Answer from the drawing. Dimensions are ordinates in mm from the lowest x, y and z of the part. A direction names the side the tool comes from. Coordinates: 2 decimals unless noted, no trailing zeros. Write each loop counter-clockwise with the first axis right and the second up, starting at its lowest first coordinate (ties: lowest second). Pieces come first, ordered by that corner, then holes.
1) Find the intervals of material crossed by line 1 (Y direction, x = 10, z = 26) (1 decimal); line 2 (Y direction, x = 1.5, z = 32); line 3 (Y direction, x = 12, z = 26), in increasing order.
2) The part is cut by section B-B (z = 20.5). Determine the outline of the cut face in (x, y) (1 decimal).
3) The part is cut by section A-A (x = 10). Determine the outline of the cut face in (y, z) (1 decimal).
4) Determine the mould class of the marked faces 1, 2, 3 and 4 for opening direction X: +X half, -X half, draft (parallel to the pull), parting line (faces both ways), or undercut.
5) Which of the six approach directions +Z, -Z, +X, -X, +Y, -Y give full straight-line access (tool end or side, diameter ignored) to the marked faces 5 and 6?
6) Each of these flat-tipped pins is pushed along its axis until it touches: pin 1 Ø2.5 at (y, z) = (9, 30.5) entering from -X; pin 2 Ø3 at (x, y) = (10, 10) entering from +Z; pin 3 Ø1.5 at (y, z) = (9, 26) entering from +X; pin 4 Ø2.5 at (x, z) = (10.5, 15) entering from +Y. Where does it stop, or does it pass through?
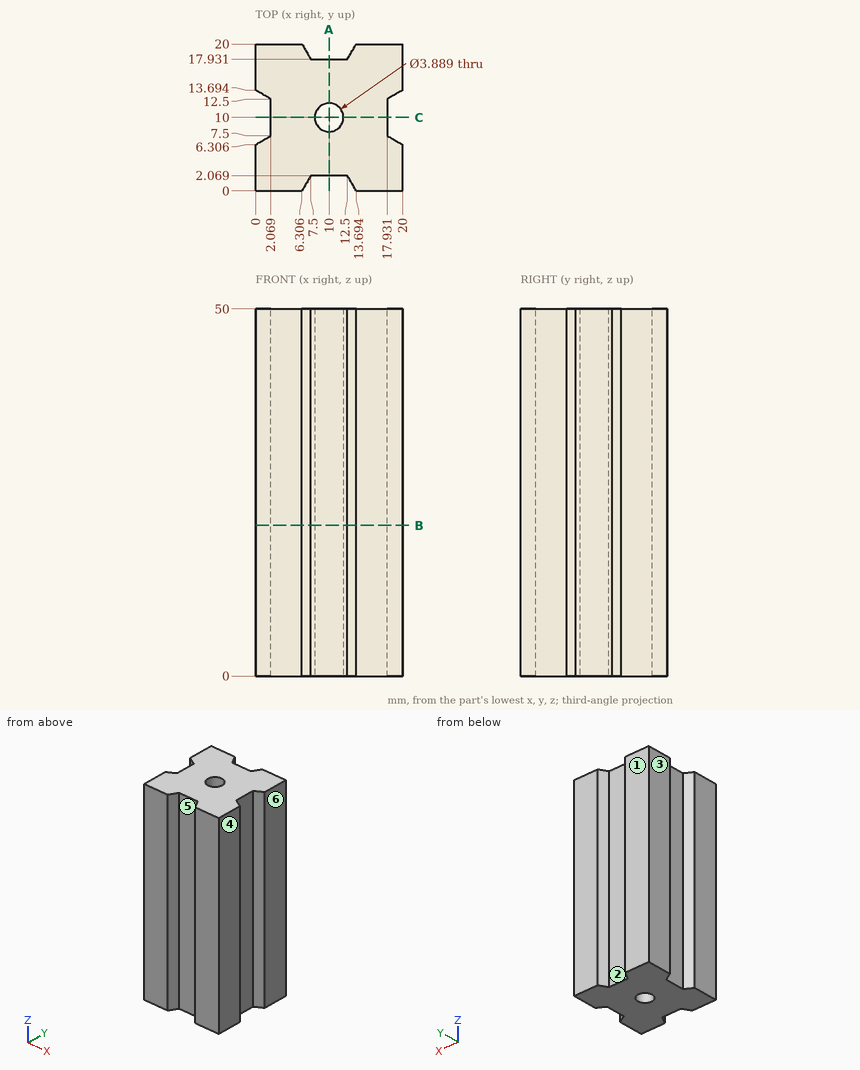
Reported:
1. line 1: y = 2.1 to 8.1, 11.9 to 17.9
1. line 2: y = 0 to 7.17, 12.83 to 20
1. line 3: y = 2.07 to 17.93
2. outline: (0, 0) - (6.3, 0) - (7.5, 2.1) - (12.5, 2.1) - (13.7, 0) - (20, 0) - (20, 6.3) - (17.9, 7.5) - (17.9, 12.5) - (20, 13.7) - (20, 20) - (13.7, 20) - (12.5, 17.9) - (7.5, 17.9) - (6.3, 20) - (0, 20) - (0, 13.7) - (2.1, 12.5) - (2.1, 7.5) - (0, 6.3) - close; hole circle Ø3.9 at (10, 10)
3. outline: (2.1, 0) - (8.1, 0) - (8.1, 50) - (2.1, 50) - close; (11.9, 0) - (17.9, 0) - (17.9, 50) - (11.9, 50) - close
4. face 1: draft
4. face 2: undercut
4. face 3: -X half
4. face 4: +X half
5. face 5: +Z, -Z, -Y
5. face 6: +Z, -Z, +X, +Y, -Y
6. pin 1: stops at x = 2.07
6. pin 2: passes through
6. pin 3: stops at x = 17.93
6. pin 4: stops at y = 17.93
